Source: CAD feature listing. Evaluate the final solid. Frame: model axes, mm. Face numbers are marked on the shaded views. A direction names the side the tool comes from. Give positions to 0.01 mm unless a question says otherwise; leave off trailing zeros. Order: outer loops, then holes, each group sorted by start corner. A loop starts at its lowest first (then second) coordinate and runs counter-clockwise, first axis right, second up.
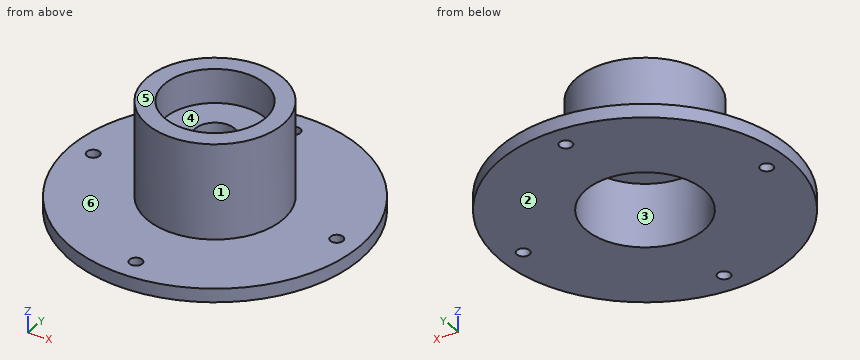
```python
from build123d import *

# Parameters (mm, degrees)
SKETCH1_W                  = 32
SKETCH1_H                  = 3
SKETCH2_R                  = 15
BOSS_EXTRUDE1_DEPTH        = 21
F_2_8_2_8_DIAMETER_HOLE1_D = 2.8


with BuildPart() as part:
    # Sketch1 → Revolve1 (revolve)
    with BuildSketch(Plane(origin=(0, 0, 0), x_dir=(1, 0, 0), z_dir=(0, 1, 0))):
        with Locations((16, -1.5)):
            Rectangle(SKETCH1_W, SKETCH1_H)
    revolve(axis=Axis((0, 0, 0), (0, 0, 1)))

    # Sketch2 → Boss-Extrude1 (add)
    with BuildSketch(Plane.XY.offset(3)):
        with Locations(Location((0, 0, 0), (0, 0, 180))):
            Circle(SKETCH2_R)
    extrude(amount=BOSS_EXTRUDE1_DEPTH)

    # Sketch3 → Cut-Revolve1 (revolve, cut)
    with BuildSketch(Plane(origin=(0, 0, 0), x_dir=(1, 0, 0), z_dir=(0, 1, 0))):
        Polygon((13, 0), (0, 0), (0, -24), (11.1, -24), (11.1, -16.5), (4.3, -16.5), (4.3, -14), (13, -14), align=None)
    revolve(axis=Axis((0, 0, 0), (0, 0, 1)), mode=Mode.SUBTRACT)

    # Ø2.8 (2.8) Diameter Hole1 (through all)
    with Locations(Plane.XY.offset(3)):
        with Locations((0, 27), (0, -27), (27, 0), (-27, 0)):
            Hole(F_2_8_2_8_DIAMETER_HOLE1_D / 2)


solid = part.part
```
1) Material intervals for L1, parallel to Y at x = 0, z = 6.5; L2, parallel to Y at x = 0, z = 18.5; L3, parallel to Z at x = 22, y = 20, sorted ascending.
Report:
L1: y = -15 to -13, 13 to 15
L2: y = -15 to -11.1, 11.1 to 15
L3: z = 0 to 3
2) Pin query (flat end, axial travel): pin 1 (8 mm diameter, centred on x = -1, y = -2, fed in from -Z); pin 2 (4.5 mm diameter, centred on x = 0, y = -27, fed in from +Z); pin 3 (12 mm diameter, centred on y = -3.5, z = 10, fed in from -X). Return the tip coordinate at first contact, or that it passes through.
Report:
pin 1: stops at z = 14
pin 2: stops at z = 3
pin 3: stops at x = -15
3) Draft query along X for the marked faces 1, 2, 3 and 4. Return one class per face: +X half, -X half, draft (parallel to the pull), parting line (faces both ways), or undercut.
Report:
face 1: parting line
face 2: draft
face 3: undercut
face 4: undercut
4) Reachability of the marked faces 5 and 6 from +Z, -Z, +X, -X, +Y, -Y: full face, straight path, thin tool, end or side. Return the list, or none.
Report:
face 5: +Z, +X, -X, +Y, -Y
face 6: +Z
5) Section query A-A, the plane x = 0. Return the cut outline in (y, z).
Report:
outline: (-32, 0) - (-28.4, 0) - (-28.4, 3) - (-32, 3) - close; (-25.6, 0) - (-13, 0) - (-13, 14) - (-4.3, 14) - (-4.3, 16.5) - (-11.1, 16.5) - (-11.1, 24) - (-15, 24) - (-15, 3) - (-25.6, 3) - close; (4.3, 14) - (13, 14) - (13, 0) - (25.6, 0) - (25.6, 3) - (15, 3) - (15, 24) - (11.1, 24) - (11.1, 16.5) - (4.3, 16.5) - close; (28.4, 0) - (32, 0) - (32, 3) - (28.4, 3) - close
6) Section query D-D, the plane z = 7.25. Return the cut outline in (x, y).
Report:
outline: circle Ø30 at (0, 0); hole circle Ø26 at (0, 0)
7) Section query B-B, the plane x = 27. Return the cut outline in (y, z).
Report:
outline: (-17.18, 0) - (-1.4, 0) - (-1.4, 3) - (-17.18, 3) - close; (1.4, 0) - (17.18, 0) - (17.18, 3) - (1.4, 3) - close
